from build123d import *

# Parameters (mm, degrees)
SKETCH1_R             = 21.5
BOSS_EXTRUDE1_DEPTH   = 17.5
CHAMFER3_SIZE         = 5
FILLET1_R             = 5
M6_TAPPED_HOLE1_D     = 5
M6_TAPPED_HOLE1_DEPTH = 17
M6_TAPPED_HOLE1_TIP   = 1.502151548
SKETCH11_R            = 2.5
CUT_EXTRUDE1_DEPTH    = 15
CHAMFER4_SIZE         = 1
SKETCH12_R            = 26
CUT_EXTRUDE2_DEPTH    = 32
M4_TAPPED_HOLE1_D     = 3.3
M4_TAPPED_HOLE1_DEPTH = 11.5
M4_TAPPED_HOLE1_TIP   = 0.991420021
CHAMFER5_SIZE         = 0.5


with BuildPart() as part:
    # Sketch1 → Boss-Extrude1 (new, symmetric)
    with BuildSketch(Plane(origin=(0, 0, 0), x_dir=(0, 0, -1), z_dir=(1, 0, 0))):
        Polygon((-40, 85), (40, 85), (40, 0), (12.5, 0), (12.5, 15), (-12.5, 15), (-12.5, 0), (-40, 0), align=None)
        with Locations((0, 54)):
            Circle(SKETCH1_R, mode=Mode.SUBTRACT)
    extrude(amount=BOSS_EXTRUDE1_DEPTH, both=True)

    # Chamfer3
    chamfer3_edges = [part.edges().sort_by_distance(p)[0] for p in [
        (0, 85, 40),
        (0, 85, -40),
    ]]
    chamfer(chamfer3_edges, length=CHAMFER3_SIZE)

    # Fillet1
    fillet1_edges = [part.edges().sort_by_distance(p)[0] for p in [
        (0, 15, -12.5),
        (0, 15, 12.5),
    ]]
    fillet(fillet1_edges, radius=FILLET1_R)

    # M6 Tapped Hole1
    with Locations(Plane(origin=(0, 0, 0), x_dir=(-1, 0, 0), z_dir=(0, -1, 0))):
        with Locations((0, -32.5), (0, 32.5)):
            Hole(M6_TAPPED_HOLE1_D / 2, depth=M6_TAPPED_HOLE1_DEPTH)
            with Locations((0, 0, -(M6_TAPPED_HOLE1_DEPTH + M6_TAPPED_HOLE1_TIP / 2))):  # 118° drill point
                Cone(0, M6_TAPPED_HOLE1_D / 2, M6_TAPPED_HOLE1_TIP, mode=Mode.SUBTRACT)

    # Sketch11 → Cut-Extrude1 (cut)
    with BuildSketch(Plane.XZ):
        with Locations(Location((0, -20, 0), (0, 0, 270))):
            Circle(SKETCH11_R)
        with BuildLine():
            Line((2.5, 20.5), (2.5, 19.5))
            ThreePointArc((2.5, 19.5), (0, 17), (-2.5, 19.5))
            Line((-2.5, 19.5), (-2.5, 20.5))
            ThreePointArc((-2.5, 20.5), (0, 23), (2.5, 20.5))
        make_face()
    extrude(amount=-CUT_EXTRUDE1_DEPTH, mode=Mode.SUBTRACT)

    # Chamfer4
    chamfer4_edges = [part.edges().sort_by_distance(p)[0] for p in [
        (0, 0, -12.5),
        (0, 0, 12.5),
    ]]
    chamfer(chamfer4_edges, length=CHAMFER4_SIZE)

    # Sketch12 → Cut-Extrude2 (cut)
    with BuildSketch(Plane.ZY.offset(17.5)):
        with Locations((0, 54)):
            Circle(SKETCH12_R)
    extrude(amount=-CUT_EXTRUDE2_DEPTH, mode=Mode.SUBTRACT)

    # M4 Tapped Hole1
    with Locations(Plane.ZY.offset(17.5)):
        with Locations((-22.5, 74), (22.5, 74), (22.5, 34), (-22.5, 34)):
            Hole(M4_TAPPED_HOLE1_D / 2, depth=M4_TAPPED_HOLE1_DEPTH)
            with Locations((0, 0, -(M4_TAPPED_HOLE1_DEPTH + M4_TAPPED_HOLE1_TIP / 2))):  # 118° drill point
                Cone(0, M4_TAPPED_HOLE1_D / 2, M4_TAPPED_HOLE1_TIP, mode=Mode.SUBTRACT)

    # Chamfer5
    chamfer5_edges = [part.edges().sort_by_distance(p)[0] for p in [
        (-17.5, 54, -26),
    ]]
    chamfer(chamfer5_edges, length=CHAMFER5_SIZE)


solid = part.part
Geometry: final body of the model. Coordinates: model frame, mm. A direction names the side the tool comes from. Coordinates: 2 decimals unless noted, no trailing zeros. Order: outer loops, then holes, each group sorted by start corner. A loop starts at its lowest first (then second) coordinate and runs counter-clockwise, first axis right, second up.
(1) First-contact query: pin 1 (4 mm diameter, centred on x = 10, z = -3, fed in from -Y); pin 2 (12 mm diameter, centred on x = -6.5, z = 3.5, fed in from -Y). Flat tips, straight axial feed; report the tip coordinate or a pass-through.
(2) Section query B-B (x = -9). Return the cut outline in (y, z), plus the area to 3 significant figures.
(3) Material intervals for probe 1 along Z at (x, y) = (-13, 34); probe 2 along Z at (x, y) = (16.65, 54); probe 3 along Z at (x, y) = (6.5, 69.5), sorted ascending.
(4) Access query for faces 1 (the face through (0, 15, 20)), 2 (the face through (0, 0, -27)), 3 (the face through (-11.67, 74.07, 24.15)), 4 (the face through (-0.25, 13.5, -11.07)). Directions: +Z, -Z, +X, -X, +Y, -Y. A direction counts if a zero-diameter tool reaches every point of the face in a straight line with its end or side. Return the directions, or none.
(5) Draft query along Y for faces 5 (the face through (15.98, 33.01, 4.66)), 6 (the face through (0, 15, 0)), 7 (the face through (1.34, 8.62, -34.61)). Return one class per face: pulls with the +Y half, pulls with the -Y half, needs draft (parallel to the pull), parting line crosses it, or undercut.
(6) Section query A-A (z = 0). Return the cut outline in (x, y).
(7) Section query C-C (x = -3.5). Return the cut outline in (y, z).
Solution:
1. pin 1: stops at y = 15
1. pin 2: stops at y = 14.58
2. outline: (0, -40) - (80, -40) - (85, -35) - (85, 35) - (80, 40) - (0, 40) - (0, 13.5) - (1, 12.5) - (10, 12.5) arc R5 cw to (15, 7.5) - (15, -7.5) arc R5 cw to (10, -12.5) - (1, -12.5) - (0, -13.5) - close; hole circle Ø52 at (54, 0); hole circle Ø3.3 at (34, -22.5); hole circle Ø3.3 at (34, 22.5); hole circle Ø3.3 at (74, -22.5); hole circle Ø3.3 at (74, 22.5)
2. area: 4,250 mm2
3. probe 1: z = -40 to -24.15, -20.85 to -16.61, 16.61 to 20.85, 24.15 to 40
3. probe 2: z = -40 to -21.5, 21.5 to 40
3. probe 3: z = -40 to -20.87, 20.87 to 40
4. face 1: -Y
4. face 2: +Z, -Z, +X, -X, -Y
4. face 3: -X
4. face 4: +X, -X, -Y
5. face 5: undercut
5. face 6: pulls with the -Y half
5. face 7: needs draft
6. outline: (-17.5, 15) - (17.5, 15) - (17.5, 32.5) - (14.5, 32.5) - (14.5, 28) - (-17, 28) - (-17.5, 27.5) - close; (-17.5, 80.5) - (-17, 80) - (14.5, 80) - (14.5, 75.5) - (17.5, 75.5) - (17.5, 85) - (-17.5, 85) - close
7. outline: (0, -40) - (80, -40) - (85, -35) - (85, 35) - (80, 40) - (0, 40) - (0, 13.5) - (1, 12.5) - (10, 12.5) arc R5 cw to (15, 7.5) - (15, -7.5) arc R5 cw to (10, -12.5) - (1, -12.5) - (0, -13.5) - close; hole circle Ø52 at (54, 0)
